Input: part model. Units: mm. Frame: model coordinates. A direction names the side the tool comes from. Round coordinates to 2 decimals unless told otherwise and drop trailing zeros. Loops run counter-clockwise (first coordinate to the right, second up) from the corner with the lowest first, then second, coordinate; pieces in that order, holes last. Notation, with made-up numbers: (85, 48.5) - (95, 48.5) arc R16 cw to (95, 58.5) - close; hole circle Ø3 at (28, -39.75). An arc over 180 degrees is marked (long way). Use CSV: the item, a comma, the result in double quotes. Start each with the question number.
1. Pin query (flat end, axial travel): P1, Ø4, axis at x = -15, y = 50, coming from the -Z side; P2, Ø3, axis at x = -56.5, y = 255, coming from the +Z side; P3, Ø5, axis at x = 0, y = -188.5, coming from the -Z side. Return the tip coordinate at first contact, or that it passes through.
2. Access query for faces 1 (the flat face through (58, 255, 4.3)), 2 (the flat face through (-1, -270, 5)). Directions: +Z, -Z, +X, -X, +Y, -Y. A direction counts if a zero-diameter tool reaches every point of the face in a straight line with its end or side. Return the directions, or none.
3. Cut plane A-A (y = -200). Return loops of the section in (x, z).
4. Pull-direction query (X, two-part tool) for faces 3 (the flat face through (-80, -4, 5)), 4 (the flat face through (-19, 4, 0)), 5 (the flat face through (-52, -255, 4.3)); classes: +X half, -X half, draft (parallel to the pull), parting line (faces both ways), or undercut.
5. Cut plane B-B (z = 2.75). Give the number of separate pieces and of enclosed holes in the cut face, and give its area (3 significant figures).
6. Material intervals for probe 1 along Y at (x, z) = (-41.3, 5); probe 2 along Y at (x, z) = (-21.5, 7.25); probe 3 along X at (y, z) = (245, 3.5), sorted ascending. Write a range as from..to.
```python
from build123d import *

# Parameters (mm, degrees)
SKETCH_1_W                = 160
SKETCH_1_H                = 540
EXTRUDE_1_DEPTH           = 10
SKETCH_2_R                = 16
CUT_EXTRUDE_1_DEPTH       = 282.780056072
SKETCH_3_R                = 18
CUT_EXTRUDE_2_DEPTH       = 282.780056072
HOLE_WIZARD_1_D           = 5.5
HOLE_WIZARD_1_CBORE_D     = 10
HOLE_WIZARD_1_CBORE_DEPTH = 5.7
HOLE_WIZARD_M5_1_D        = 4.2
HOLE_WIZARD_M5_2_D        = 4.2
HOLE_WIZARD_M5_3_D        = 4.2
HOLE_WIZARD_M3_1_D        = 2.5
HOLE_WIZARD_M6_2_D        = 5
CUT_EXTRUDE_3_DEPTH       = 5.7
CUT_EXTRUDE_4_DEPTH       = 282.660238585
HOLE_WIZARD_M6_3_D        = 5


with BuildPart() as part:
    # 草图1 → 凸台-拉伸1 (new body)
    with BuildSketch(Plane.XY):
        Rectangle(SKETCH_1_W, SKETCH_1_H)
    extrude(amount=EXTRUDE_1_DEPTH)

    # 草图2 → 切除-拉伸1 (cut, through all)
    with BuildSketch(Plane.XY.offset(10)):
        with Locations((0, 190)):
            Circle(SKETCH_2_R)
        with Locations((0, -210)):
            Circle(SKETCH_2_R)
    extrude(amount=-CUT_EXTRUDE_1_DEPTH, mode=Mode.SUBTRACT)

    # 草图3 → 切除-拉伸2 (cut, through all)
    with BuildSketch(Plane.XY.offset(10)):
        Circle(SKETCH_3_R)
    extrude(amount=-CUT_EXTRUDE_2_DEPTH, mode=Mode.SUBTRACT)

    # 打孔尺寸根据内六角圆柱头螺钉的类型1 (through all)
    with Locations(Plane.XY.offset(10)):
        with Locations((-55, 255), (55, 255), (55, -255), (-55, -255)):
            CounterBoreHole(HOLE_WIZARD_1_D / 2, HOLE_WIZARD_1_CBORE_D / 2, HOLE_WIZARD_1_CBORE_DEPTH)

    # M5 螺纹孔1 (through all)
    with Locations(Plane.XY.offset(10)):
        with Locations((0, 211.5)):
            Hole(HOLE_WIZARD_M5_1_D / 2)

    # M5 螺纹孔2 (through all)
    with Locations(Plane.XY.offset(10)):
        with Locations((0, -231.5)):
            Hole(HOLE_WIZARD_M5_2_D / 2)

    # M5 螺纹孔3 (through all)
    with Locations(Plane.XY.offset(10)):
        with Locations((21.5, -210), (-21.5, -210), (0, -188.5), (-21.5, 190), (21.5, 190), (0, 168.5)):
            Hole(HOLE_WIZARD_M5_3_D / 2)

    # M3 螺纹孔1 (through all)
    with Locations(Plane.XY.offset(10)):
        with Locations((-41.3, 265), (-41.3, 245)):
            Hole(HOLE_WIZARD_M3_1_D / 2)

    # M6 螺纹孔2 (through all)
    with Locations(Plane(origin=(0, 0, 0), x_dir=(-1, 0, 0), z_dir=(0, 0, -1))):
        with Locations((-50, 15), (-50, -15), (50, 15), (50, -15)):
            Hole(HOLE_WIZARD_M6_2_D / 2)

    # 草图24 → 切除-拉伸3 (cut)
    with BuildSketch(Plane.XY.offset(10)):
        with BuildLine():
            Line((-50, 260), (-50, 250))
            ThreePointArc((-50, 250), (-55, 245), (-60, 250))
            Line((-60, 250), (-60, 260))
            ThreePointArc((-60, 260), (-55, 265), (-50, 260))
        make_face()
        with BuildLine():
            Line((60, 260), (60, 250))
            ThreePointArc((60, 250), (55, 245), (50, 250))
            Line((50, 250), (50, 260))
            ThreePointArc((50, 260), (55, 265), (60, 260))
        make_face()
        with BuildLine():
            Line((-50, -250), (-50, -260))
            ThreePointArc((-50, -260), (-55, -265), (-60, -260))
            Line((-60, -260), (-60, -250))
            ThreePointArc((-60, -250), (-55, -245), (-50, -250))
        make_face()
        with BuildLine():
            Line((60, -250), (60, -260))
            ThreePointArc((60, -260), (55, -265), (50, -260))
            Line((50, -260), (50, -250))
            ThreePointArc((50, -250), (55, -245), (60, -250))
        make_face()
    extrude(amount=-CUT_EXTRUDE_3_DEPTH, mode=Mode.SUBTRACT)

    # 草图25 → 切除-拉伸4 (cut, through all)
    with BuildSketch(Plane.XY.offset(4.3)):
        with BuildLine():
            Line((-52.25, 260), (-52.25, 250))
            ThreePointArc((-52.25, 250), (-55, 247.25), (-57.75, 250))
            Line((-57.75, 250), (-57.75, 260))
            ThreePointArc((-57.75, 260), (-55, 262.75), (-52.25, 260))
        make_face()
        with BuildLine():
            Line((57.75, 260), (57.75, 250))
            ThreePointArc((57.75, 250), (55, 247.25), (52.25, 250))
            Line((52.25, 250), (52.25, 260))
            ThreePointArc((52.25, 260), (55, 262.75), (57.75, 260))
        make_face()
        with BuildLine():
            Line((-52.25, -250), (-52.25, -260))
            ThreePointArc((-52.25, -260), (-55, -262.75), (-57.75, -260))
            Line((-57.75, -260), (-57.75, -250))
            ThreePointArc((-57.75, -250), (-55, -247.25), (-52.25, -250))
        make_face()
        with BuildLine():
            Line((57.75, -250), (57.75, -260))
            ThreePointArc((57.75, -260), (55, -262.75), (52.25, -260))
            Line((52.25, -260), (52.25, -250))
            ThreePointArc((52.25, -250), (55, -247.25), (57.75, -250))
        make_face()
    extrude(amount=-CUT_EXTRUDE_4_DEPTH, mode=Mode.SUBTRACT)

    # M6 螺纹孔3 (through all)
    with Locations(Plane(origin=(0, 0, 0), x_dir=(-1, 0, 0), z_dir=(0, 0, -1))):
        with Locations((15, -50), (-15, -50), (-15, 50), (15, 50)):
            Hole(HOLE_WIZARD_M6_3_D / 2)


solid = part.part
```
Established:
1,P1,"passes through"
1,P2,"stops at z = 4.3"
1,P3,"stops at z = 0"
2,face 1,"+Z"
2,face 2,"+Z, -Z, +X, -X, -Y"
3,outline,"(-80, 0) - (-12.49, 0) - (-12.49, 10) - (-80, 10) - close; (12.49, 0) - (80, 0) - (80, 10) - (12.49, 10) - close"
4,face 3,"-X half"
4,face 4,"draft"
4,face 5,"undercut"
5,separate pieces,"1"
5,enclosed holes,"25"
5,area,"83,200 mm2"
6,probe 1,"y = -270..243.75, 246.25..263.75, 266.25..270"
6,probe 2,"y = -270..-212.1, -207.9..187.9, 192.1..270"
6,probe 3,"x = -80..-42.55, -40.05..80"
